For this review, use the dimensioned drawing (mm, ordinates from the lowest corner) and the shaded views. A direction names the side the tool comes from. Give positions to 0.01 mm unless a question says otherwise; leave off trailing zeros. Write each loop counter-clockwise with the first axis right and the second up, starting at its lowest first coordinate (ties: lowest second). Pieces come first, ordered by that corner, then holes. Notation, with made-up numbers: M 45.5,-35.5 L 91.5,-35.5 A27 cw 91.5,-18.5 Z; hole C 88.5,-24 d5. An arc over 180 degrees is marked long. Answer in a Markdown table with one row per item.
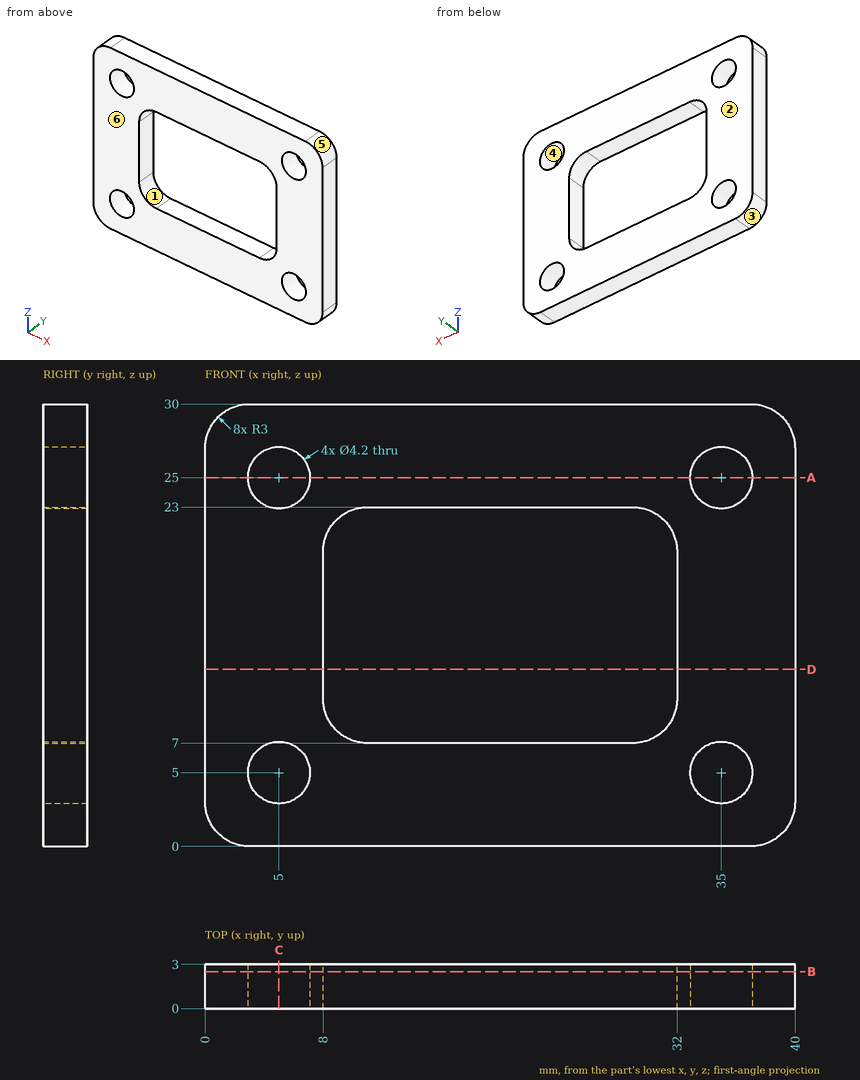
1) Add section B-B (y = 2.5). Write out the cut boundary in (x, z), and give its area (3 significant figures).
Geometry says:
| item | result |
|---|---|
| outline | M 0,3 A3 ccw 3,0 L 37,0 A3 ccw 40,3 L 40,27 A3 ccw 37,30 L 3,30 A3 ccw 0,27 Z; hole C 5,5 d4.2; hole C 5,25 d4.2; hole M 8,10 A3 ccw 11,7 L 29,7 A3 ccw 32,10 L 32,20 A3 ccw 29,23 L 11,23 A3 ccw 8,20 Z; hole C 35,5 d4.2; hole C 35,25 d4.2 |
| area | 761 mm^2 |
2) To check wall thickness, follow probe 1 along X at (y, z) = (2.05, 25); probe 2 along X at (y, z) = (1, 17); probe 3 along X at (y, z) = (0.2, 4.5). State the ranges of each line that lie inside material, in increasing order. Write a range as [from, to].
Geometry says:
| item | result |
|---|---|
| probe 1 | [0, 2.9], [7.1, 32.9], [37.1, 40] |
| probe 2 | [0, 8], [32, 40] |
| probe 3 | [0, 2.96], [7.04, 32.96], [37.04, 40] |
3) Add section D-D (z = 12). Write out the cut boundary in (x, y).
Geometry says:
| item | result |
|---|---|
| outline | M 0,0 L 8,0 L 8,3 L 0,3 Z; M 32,0 L 40,0 L 40,3 L 32,3 Z |
4) Add section A-A (z = 25). Write out the cut boundary in (x, y).
Geometry says:
| item | result |
|---|---|
| outline | M 0,0 L 2.9,0 L 2.9,3 L 0,3 Z; M 7.1,0 L 32.9,0 L 32.9,3 L 7.1,3 Z; M 37.1,0 L 40,0 L 40,3 L 37.1,3 Z |
5) Add section C-C (x = 5). Write out the cut boundary in (y, z), and give its area (3 significant figures).
Geometry says:
| item | result |
|---|---|
| outline | M 0,0 L 3,0 L 3,2.9 L 0,2.9 Z; M 0,7.1 L 3,7.1 L 3,22.9 L 0,22.9 Z; M 0,27.1 L 3,27.1 L 3,30 L 0,30 Z |
| area | 64.8 mm^2 |
6) The part is to be moulded in two halves that separate along X. For the marked faces 3, 4, 5 and 6, say which applies: released by +X, released by -X, zero draft, split by the parting line, or undercut.
Geometry says:
| item | result |
|---|---|
| face 3 | released by -X |
| face 4 | undercut |
| face 5 | released by +X |
| face 6 | zero draft |
7) For the marked faces 1 and 2, list the 3-axis set-ups (+Z, -Z, +X, -X, +Y, -Y) from which the entire face can be reached by the end or side of a thin tool; tool diameter is ignored.
Geometry says:
| item | result |
|---|---|
| face 1 | +Y, -Y |
| face 2 | +Z, -Z, +X, -X, +Y |
8) Insertion check: P1, Ø2.5, axis at x = 35, z = 25, coming from the -Y side. The pin has a flat end and moves straight along its axis. Give the tip position at first contact, or say it passes through.
Geometry says:
| item | result |
|---|---|
| P1 | through |
